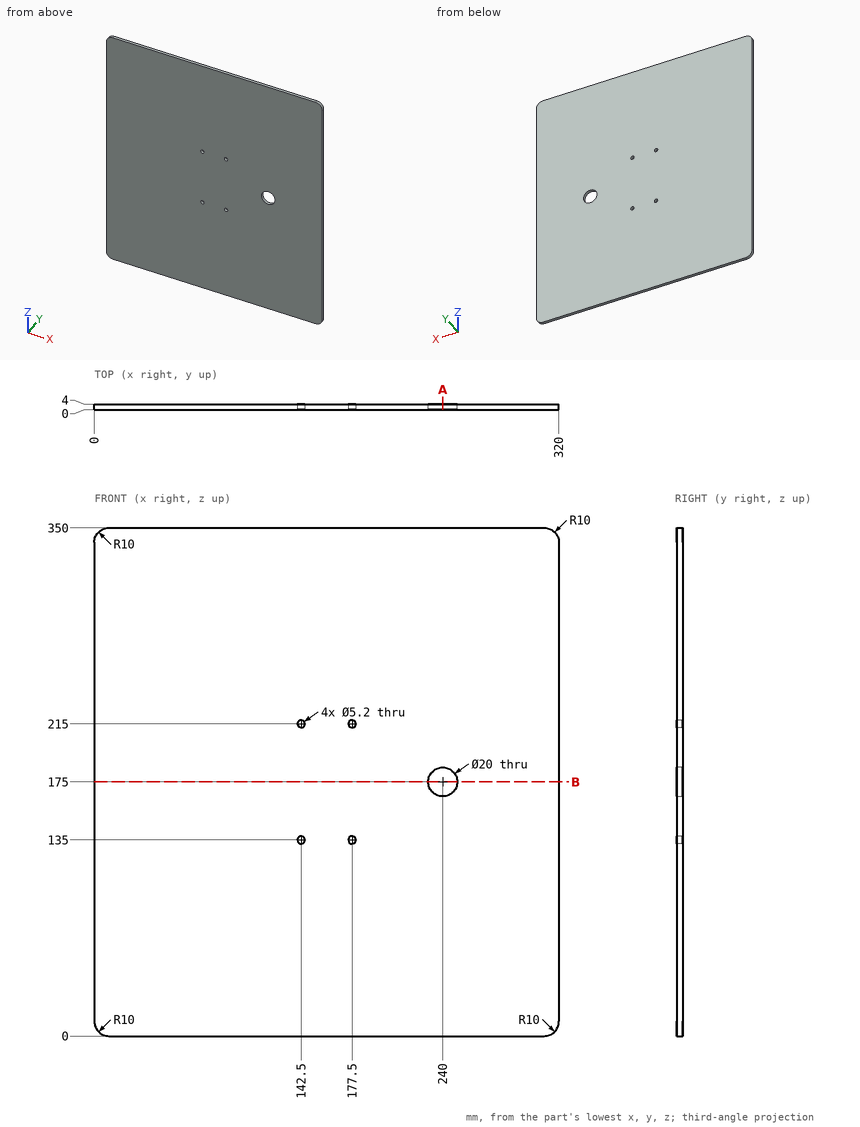
Geometry: see drawing. Coordinates: mm, zero at the bounding-box minimum. Round coordinates to 2 decimals unless told otherwise and drop trailing zeros. Order: outer loops, then holes, each group sorted by start corner. A loop starts at its lowest first (then second) coordinate and runs counter-clockwise, first axis right, second up. Notation, with made-up numbers: (37.25, 6) - (54.25, 6) arc R25 ccw to (54.25, 38) - close; hole circle Ø2 at (23, 75). An arc over 180 degrees is marked (long way). One line per question, with ' | ' between items. Start each with the question number.
1) Cut plane A-A, the plane x = 240. Return the cut outline in (y, z), then the cut area to 3 significant figures.
2) Cut plane B-B, the plane z = 175. Return the cut outline in (x, y).
3) Ray query, probe 1 along X at (y, z) = (2.5, 215); probe 2 along Z at (x, y) = (177.5, 2.15); probe 3 along X at (y, z) = (1.7, 175). Return the intervals inside material, ascending.
4) Contact query for a flat-ended pin moving along its axis: P1, Ø4.5, axis at x = 142.5, z = 135, coming from the -Y side. Output: stop coordinate, or through.
Worked out:
1) outline: (0, 0) - (4, 0) - (4, 165) - (0, 165) - close; (0, 185) - (4, 185) - (4, 350) - (0, 350) - close | area: 1,320 mm^2
2) outline: (0, 0) - (230, 0) - (230, 4) - (0, 4) - close; (250, 0) - (320, 0) - (320, 4) - (250, 4) - close
3) probe 1: x = 0 to 139.9, 145.1 to 174.9, 180.1 to 320 | probe 2: z = 0 to 132.4, 137.6 to 212.4, 217.6 to 350 | probe 3: x = 0 to 230, 250 to 320
4) P1: passes through
